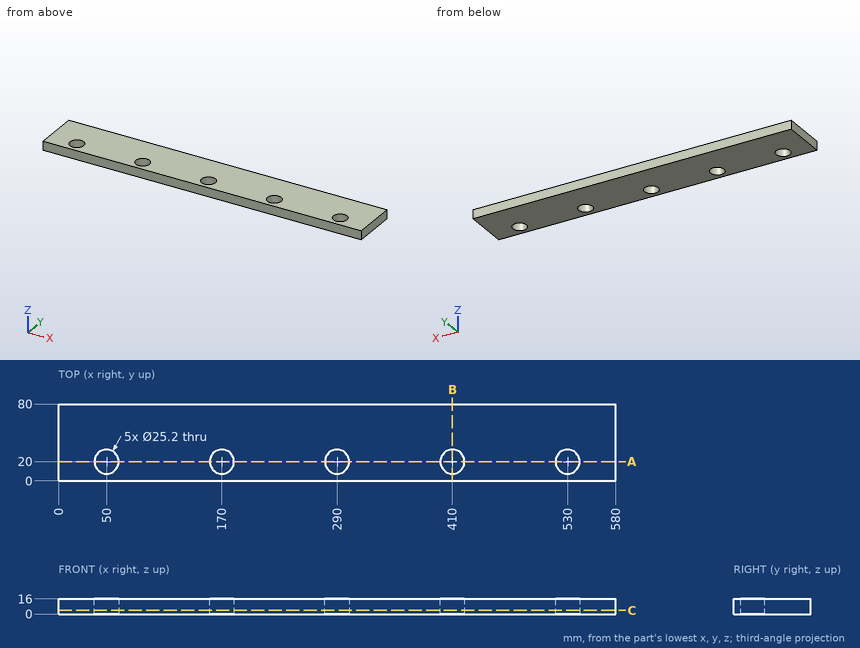
Print and shaded views of the part. All mm, measured from the part's lowest x, y and z. Coordinates: 2 decimals unless noted, no trailing zeros. Loops run counter-clockwise (first coordinate to the right, second up) from the corner with the lowest first, then second, coordinate; pieces in that order, holes last. Notation, with made-up numbers: (36.25, 76.25) - (72.25, 76.25) arc R9 cw to (72.25, 86.25) - close; hole circle Ø6 at (21, 55). An arc over 180 degrees is marked (long way). Write item = value, one per line. Start each with the question number.
Item 1: Saw through at C-C, the plane z = 4. List the corners of the cut face in (x, y).
Item 2: Saw through at B-B, the plane x = 410. List the corners of the cut face in (y, z).
Item 3: Wall check: probe 1 along Y at (x, z) = (290, 12.75); probe 2 along X at (y, z) = (31, 10.5); probe 3 along X at (y, z) = (11.5, 12.75). Give the ranges that are in metal, low to high. Write a range as [from, to].
Item 4: Saw through at A-A, the plane y = 20. List the corners of the cut face in (x, z), then the cut area to 3 significant figures.
Item 5: Drop a flat-ended pin along its axis: pin 1 Ø6 at (x, y) = (100.5, 39.5) entering from -Z. Give the stop position or say it passes through.
Answers:
q1.outline = (0, 0) - (580, 0) - (580, 80) - (0, 80) - close; hole circle Ø25.2 at (50, 20); hole circle Ø25.2 at (170, 20); hole circle Ø25.2 at (290, 20); hole circle Ø25.2 at (410, 20); hole circle Ø25.2 at (530, 20)
q2.outline = (0, 0) - (7.4, 0) - (7.4, 16) - (0, 16) - close; (32.6, 0) - (80, 0) - (80, 16) - (32.6, 16) - close
q3.probe_1 = [0, 7.4], [32.6, 80]
q3.probe_2 = [0, 43.86], [56.14, 163.86], [176.14, 283.86], [296.14, 403.86], [416.14, 523.86], [536.14, 580]
q3.probe_3 = [0, 40.7], [59.3, 160.7], [179.3, 280.7], [299.3, 400.7], [419.3, 520.7], [539.3, 580]
q4.outline = (0, 0) - (37.4, 0) - (37.4, 16) - (0, 16) - close; (62.6, 0) - (157.4, 0) - (157.4, 16) - (62.6, 16) - close; (182.6, 0) - (277.4, 0) - (277.4, 16) - (182.6, 16) - close; (302.6, 0) - (397.4, 0) - (397.4, 16) - (302.6, 16) - close; (422.6, 0) - (517.4, 0) - (517.4, 16) - (422.6, 16) - close; (542.6, 0) - (580, 0) - (580, 16) - (542.6, 16) - close
q4.area = 7,260 mm2
q5.pin_1 = 0
